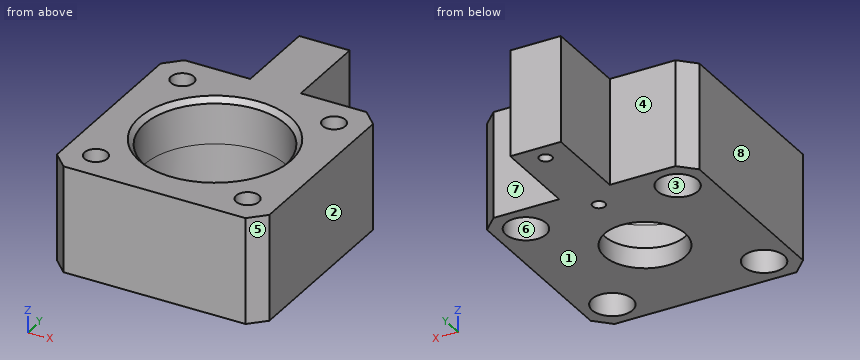
from build123d import *

# Parameters (mm, degrees)
SKETCH_1_W                = 42
SKETCH_1_H                = 42
EXTRUDE_1_DEPTH           = 12
SKETCH_2_R                = 14
CUT_EXTRUDE_1_DEPTH       = 8
SKETCH_3_R                = 8
CUT_EXTRUDE_2_DEPTH       = 50.629250448
CHAMFER_1_SIZE            = 3
HOLE_WIZARD_2_D           = 4.5
HOLE_WIZARD_2_CBORE_D     = 8
HOLE_WIZARD_2_CBORE_DEPTH = 4.6
EXTRUDE_START             = 9
SKETCH_10_R               = 2.25
SKETCH_10_R_2             = 14
EXTRUDE_2_DEPTH           = 9
SKETCH_11_W               = 10
SKETCH_11_H               = 17
EXTRUDE_3_DEPTH           = 21
HOLE_WIZARD_M3_1_D        = 2.5
HOLE_WIZARD_M3_1_DEPTH    = 7
HOLE_WIZARD_M3_1_TIP      = 0.751075774
CHAMFER_2_SIZE            = 1


with BuildPart() as part:
    # 草图1 → 凸台-拉伸1 (new body)
    with BuildSketch(Plane.XY):
        with Locations((0, 23.25)):
            Rectangle(SKETCH_1_W, SKETCH_1_H)
    extrude(amount=EXTRUDE_1_DEPTH)

    # 草图2 → 切除-拉伸1 (cut)
    with BuildSketch(Plane.XY.offset(12)):
        with Locations((0, 23.25)):
            Circle(SKETCH_2_R)
    extrude(amount=-CUT_EXTRUDE_1_DEPTH, mode=Mode.SUBTRACT)

    # 草图3 → 切除-拉伸2 (cut, through all)
    with BuildSketch(Plane.XY.offset(4)):
        with Locations((0, 23.25)):
            Circle(SKETCH_3_R)
    extrude(amount=-CUT_EXTRUDE_2_DEPTH, mode=Mode.SUBTRACT)

    # 倒角1
    chamfer_1_edges = [part.edges().sort_by_distance(p)[0] for p in [
        (21, 2.25, 6),
        (-21, 2.25, 6),
        (-21, 44.25, 6),
        (21, 44.25, 6),
    ]]
    chamfer(chamfer_1_edges, length=CHAMFER_1_SIZE)

    # 打孔尺寸根据内六角圆柱头螺钉的类型2 (through all)
    with Locations(Plane(origin=(0, 0, 0), x_dir=(-1, 0, 0), z_dir=(0, 0, -1))):
        with Locations((-15, 38.25), (15, 38.25), (15, 8.25), (-15, 8.25)):
            CounterBoreHole(HOLE_WIZARD_2_D / 2, HOLE_WIZARD_2_CBORE_D / 2, HOLE_WIZARD_2_CBORE_DEPTH)

    # 草图10 → 凸台-拉伸2 (add)
    with BuildSketch(Plane.XY.offset(12).offset(EXTRUDE_START)):
        Polygon((-18, 2.25), (18, 2.25), (21, 5.25), (21, 41.25), (18, 44.25), (-18, 44.25), (-21, 41.25), (-21, 5.25), align=None)
        with Locations(Location((-15, 38.25, 0), (0, 0, 180))):
            Circle(SKETCH_10_R, mode=Mode.SUBTRACT)
        with Locations((0, 23.25)):
            Circle(SKETCH_10_R_2, mode=Mode.SUBTRACT)
        with Locations(Location((15, 38.25, 0), (0, 0, 180))):
            Circle(SKETCH_10_R, mode=Mode.SUBTRACT)
        with Locations(Location((15, 8.25, 0), (0, 0, 180))):
            Circle(SKETCH_10_R, mode=Mode.SUBTRACT)
        with Locations(Location((-15, 8.25, 0), (0, 0, 180))):
            Circle(SKETCH_10_R, mode=Mode.SUBTRACT)
    extrude(amount=-EXTRUDE_2_DEPTH)

    # 草图11 → 凸台-拉伸3 (add)
    with BuildSketch(Plane(origin=(0, 0, 0), x_dir=(-1, 0, 0), z_dir=(0, 0, -1))):
        with Locations((0, 52.75)):
            Rectangle(SKETCH_11_W, SKETCH_11_H)
    extrude(amount=-EXTRUDE_3_DEPTH)

    # M3 螺纹孔1
    with Locations(Plane(origin=(0, 0, 0), x_dir=(-1, 0, 0), z_dir=(0, 0, -1))):
        with Locations((0, 57.75), (0, 39.25)):
            Hole(HOLE_WIZARD_M3_1_D / 2, depth=HOLE_WIZARD_M3_1_DEPTH)
            with Locations((0, 0, -(HOLE_WIZARD_M3_1_DEPTH + HOLE_WIZARD_M3_1_TIP / 2))):  # 118° drill point
                Cone(0, HOLE_WIZARD_M3_1_D / 2, HOLE_WIZARD_M3_1_TIP, mode=Mode.SUBTRACT)

    # 倒角2
    chamfer_2_edges = [part.edges().sort_by_distance(p)[0] for p in [
        (-14, 23.25, 21),
    ]]
    chamfer(chamfer_2_edges, length=CHAMFER_2_SIZE)


solid = part.part
The model under review builds one solid part; all positions refer to its coordinate system, in mm. Face numbers are marked on the shaded views. A direction names the side the tool comes from. Coordinates: 2 decimals unless noted, no trailing zeros. Order: outer loops, then holes, each group sorted by start corner. A loop starts at its lowest first (then second) coordinate and runs counter-clockwise, first axis right, second up. Notation, with made-up numbers: (79, 74.5) -> (113, 74.5) arc R24 cw to (113, 108.5) -> close; hole circle Ø9 at (86.25, 4). An arc over 180 degrees is marked (long way). Answer in a Markdown table with one row per item.
(1) The part is to be moulded in two halves that separate along X. For the marked faces 1, 2 and 3, say which applies: +X half, -X half, draft (parallel to the pull), parting line (faces both ways), or undercut.
Answers:
| item | result |
|---|---|
| face 1 | draft |
| face 2 | +X half |
| face 3 | undercut |
(2) Insertion check: pin 1 (4 mm diameter, centred on x = 14, y = 8.5, fed in from -Z); pin 2 (4 mm diameter, centred on x = 15, y = 38.25, fed in from +Z); pin 3 (8 mm diameter, centred on y = 49.5, z = 5, fed in from +X). Each pin has a flat end and moves straight along its axis. Give the tip position at first contact, or say it passes through.
Answers:
| item | result |
|---|---|
| pin 1 | z = 4.6 |
| pin 2 | through |
| pin 3 | x = 5 |
(3) Consider section B-B (z = 15.25). Write out the cut boundary in (x, y).
Answers:
| item | result |
|---|---|
| outline | (-21, 5.25) -> (-18, 2.25) -> (18, 2.25) -> (21, 5.25) -> (21, 41.25) -> (18, 44.25) -> (5, 44.25) -> (5, 61.25) -> (-5, 61.25) -> (-5, 44.25) -> (-18, 44.25) -> (-21, 41.25) -> close; hole circle Ø4.5 at (-15, 8.25); hole circle Ø4.5 at (-15, 38.25); hole circle Ø28 at (0, 23.25); hole circle Ø4.5 at (15, 8.25); hole circle Ø4.5 at (15, 38.25) |
(4) Consider section C-C (y = 48.5). Write out the cut boundary in (x, z), plus the area to 3 significant figures.
Answers:
| item | result |
|---|---|
| outline | (-5, 0) -> (5, 0) -> (5, 21) -> (-5, 21) -> close |
| area | 210 mm² |
(5) Machinability: for the marked faces 4, 5, 6, 7 and 8, which of the approach directions +Z, -Z, +X, -X, +Y, -Y give a long, thin tool a straight path to every point of the face, cutting with its end or side? Answer none if there is none.
Answers:
| item | result |
|---|---|
| face 4 | +Z, -Z, -X, +Y |
| face 5 | +Z, -Z, +X, -Y |
| face 6 | -Z |
| face 7 | +Z, -Z, +X, +Y |
| face 8 | +Z, -Z, -X, +Y, -Y |
(6) Consider section A-A (y = 23.25). Write out the cut boundary in (x, z).
Answers:
| item | result |
|---|---|
| outline | (-21, 0) -> (-8, 0) -> (-8, 4) -> (-14, 4) -> (-14, 20) -> (-15, 21) -> (-21, 21) -> close; (8, 0) -> (21, 0) -> (21, 21) -> (15, 21) -> (14, 20) -> (14, 4) -> (8, 4) -> close |
(7) Wall thickness on line 1 along Y through (x, z) = (0, 5); line 2 along Y through (x, z) = (15, 9.25); line 3 along X through (y, z) = (8.25, 7.5): over which ranges is each line inside the solid? List them lowest first.
Answers:
| item | result |
|---|---|
| line 1 | 2.25 to 9.25, 37.25 to 38, 40.5 to 56.5, 59 to 61.25 |
| line 2 | 2.25 to 6, 10.5 to 36, 40.5 to 44.25 |
| line 3 | -21 to -17.25, -12.75 to 12.75, 17.25 to 21 |
